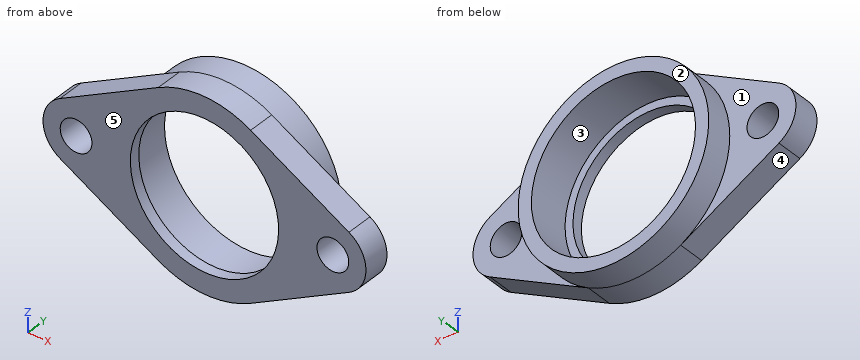
```python
from build123d import *

# Parameters (mm, degrees)
SKETCH_1_R          = 6
EXTRUDE_1_DEPTH     = 10
SKETCH_2_R          = 36
EXTRUDE_2_DEPTH     = 10
SKETCH_3_R          = 31
CUT_EXTRUDE_1_DEPTH = 16
SKETCH_4_R          = 28
CUT_EXTRUDE_2_DEPTH = 16


with BuildPart() as part:
    # 草图1 → 凸台-拉伸1 (new body)
    with BuildSketch(Plane(origin=(0, 0, 0), x_dir=(1, 0, 0), z_dir=(0, 1, 0))):
        with BuildLine():
            Line((-54.556701031, 10.934640946), (-17.443298969, 31.491765925))
            ThreePointArc((-17.443298969, 31.491765925), (0, 36), (17.443298969, 31.491765925))
            Line((17.443298969, 31.491765925), (54.556701031, 10.934640946))
            ThreePointArc((54.556701031, 10.934640946), (61, 0), (54.556701031, -10.934640946))
            Line((54.556701031, -10.934640946), (17.443298969, -31.491765925))
            ThreePointArc((17.443298969, -31.491765925), (0, -36), (-17.443298969, -31.491765925))
            Line((-17.443298969, -31.491765925), (-54.556701031, -10.934640946))
            ThreePointArc((-54.556701031, -10.934640946), (-61, 0), (-54.556701031, 10.934640946))
        make_face()
        with Locations(Location((48.5, 0, 0), (0, 0, 270))):
            Circle(SKETCH_1_R, mode=Mode.SUBTRACT)
        with Locations(Location((-48.5, 0, 0), (0, 0, 270))):
            Circle(SKETCH_1_R, mode=Mode.SUBTRACT)
    extrude(amount=EXTRUDE_1_DEPTH)

    # 草图2 → 凸台-拉伸2 (add)
    with BuildSketch(Plane(origin=(0, 10, 0), x_dir=(1, 0, 0), z_dir=(0, 1, 0))):
        with Locations(Location((0, 0, 0), (0, 0, 118.982082268))):
            Circle(SKETCH_2_R)
    extrude(amount=EXTRUDE_2_DEPTH)

    # 草图3 → 切除-拉伸1 (cut)
    with BuildSketch(Plane(origin=(0, 20, 0), x_dir=(1, 0, 0), z_dir=(0, 1, 0))):
        with Locations(Location((0, 0, 0), (0, 0, 270))):
            Circle(SKETCH_3_R)
    extrude(amount=-CUT_EXTRUDE_1_DEPTH, mode=Mode.SUBTRACT)

    # 草图4 → 切除-拉伸2 (cut)
    with BuildSketch(Plane(origin=(0, 4, 0), x_dir=(1, 0, 0), z_dir=(0, 1, 0))):
        with Locations(Location((0, 0, 0), (0, 0, 270))):
            Circle(SKETCH_4_R)
    extrude(amount=-CUT_EXTRUDE_2_DEPTH, mode=Mode.SUBTRACT)


solid = part.part
```
Input: part model. Units: mm. Frame: model coordinates. Face numbers are marked on the shaded views. A direction names the side the tool comes from. Coordinates: 2 decimals unless noted, no trailing zeros. Loops run counter-clockwise (first coordinate to the right, second up) from the corner with the lowest first, then second, coordinate; pieces in that order, holes last. Notation, with made-up numbers: M -4,54 L 22,54 A19 ccw 22,80 Z; hole C -13.5,-25 d6. An arc over 180 degrees is marked long. One line per item, written item: value.
(1) Line query: line 1 along X through (y, z) = (6, 0); line 2 along X through (y, z) = (2.5, 0); line 3 along X through (y, z) = (12.5, 0). Output: solid intervals per line, ascending. Write a range as from..to.
Filled in:
line 1: -61..-54.5, -42.5..-31, 31..42.5, 54.5..61
line 2: -61..-54.5, -42.5..-28, 28..42.5, 54.5..61
line 3: -36..-31, 31..36
(2) Pull-direction query (X, two-part tool) for the marked faces 3, 4 and 5; classes: +X half, -X half, draft (parallel to the pull), parting line (faces both ways), or undercut.
Filled in:
face 3: undercut
face 4: -X half
face 5: draft
(3) Reachability of the marked faces 1 and 2 from +Z, -Z, +X, -X, +Y, -Y: full face, straight path, thin tool, end or side. Return the list, or none.
Filled in:
face 1: -X, +Y
face 2: +Z, -Z, +X, -X, +Y
(4) Section A-A (y = 6.75). Output: boundary loops of the cut face in (x, z).
Filled in:
outline: M -54.56,-10.93 L -17.44,-31.49 A36 ccw 17.44,-31.49 L 54.56,-10.93 A12.5 ccw 54.56,10.93 L 17.44,31.49 A36 ccw -17.44,31.49 L -54.56,10.93 A12.5 ccw Z; hole C -48.5,0 d12; hole C 0,0 d62; hole C 48.5,0 d12
(5) Pin query (flat end, axial travel): pin 1 (12 mm diameter, centred on x = 16, z = 8.5, fed in from +Y) (3 decimals); pin 2 (5 mm diameter, centred on y = 5.5, z = 10.5, fed in from -X); pin 3 (10 mm diameter, centred on y = 7.5, z = -9.5, fed in from -X); pin 4 (13 mm diameter, centred on x = 42, z = -7.5, fed in from +Y). Return the tip coordinate at first contact, or that it passes through.
Filled in:
pin 1: through
pin 2: x = -58.1
pin 3: x = -60.16
pin 4: y = 10
(6) Section C-C (x = -13.5). Output: boundary loops of the cut face in (y, z), and give its area (3 significant figures).
Filled in:
outline: M 0,-33.37 L 20,-33.37 L 20,-27.91 L 4,-27.91 L 4,-24.53 L 0,-24.53 Z; M 0,24.53 L 4,24.53 L 4,27.91 L 20,27.91 L 20,33.37 L 0,33.37 Z
area: 246 mm^2
(7) Section D-D (z = 17.5). Output: boundary loops of the cut face in (x, y), and give its area (3 significant figures).
Filled in:
outline: M -42.7,0 L -21.86,0 L -21.86,4 L -25.59,4 L -25.59,20 L -31.46,20 L -31.46,10 L -42.7,10 Z; M 21.86,0 L 42.7,0 L 42.7,10 L 31.46,10 L 31.46,20 L 25.59,20 L 25.59,4 L 21.86,4 Z
area: 490 mm^2
(8) Section B-B (z = 0). Output: boundary loops of the cut face in (x, y), and give its area (3 significant figures).
Filled in:
outline: M -61,0 L -54.5,0 L -54.5,10 L -61,10 Z; M -42.5,0 L -28,0 L -28,4 L -31,4 L -31,20 L -36,20 L -36,10 L -42.5,10 Z; M 28,0 L 42.5,0 L 42.5,10 L 36,10 L 36,20 L 31,20 L 31,4 L 28,4 Z; M 54.5,0 L 61,0 L 61,10 L 54.5,10 Z
area: 484 mm^2
